```python
from build123d import *

# Parameters (mm, degrees)
SKETCH_1_W            = 100
SKETCH_1_H            = 50
EXTRUDE_1_DEPTH       = 15
HOLE_WIZARD_7_0_7_1_D = 7
CHAMFER_1_SIZE        = 3
SKETCH_6_W            = 2
SKETCH_6_H            = 30
CUT_EXTRUDE_1_DEPTH   = 113


with BuildPart() as part:
    # 草图1 → 凸台-拉伸1 (new body)
    with BuildSketch(Plane.XY):
        with Locations((50, 25)):
            Rectangle(SKETCH_1_W, SKETCH_1_H)
    extrude(amount=EXTRUDE_1_DEPTH)

    # Ø7.0 (7) 直径孔1 (through all)
    with Locations(Plane(origin=(0, 0, 0), x_dir=(-1, 0, 0), z_dir=(0, 0, -1))):
        with Locations((-10, 44), (-10, 6), (-90, 44), (-90, 6)):
            Hole(HOLE_WIZARD_7_0_7_1_D / 2)

    # 倒角1
    chamfer_1_edges = [part.edges().sort_by_distance(p)[0] for p in [
        (0, 50, 7.5),
        (100, 50, 7.5),
        (100, 0, 7.5),
        (0, 0, 7.5),
    ]]
    chamfer(chamfer_1_edges, length=CHAMFER_1_SIZE)

    # 草图6 → 切除-拉伸1 (cut)
    with BuildSketch(Plane.ZY):
        with Locations((1, 25)):
            Rectangle(SKETCH_6_W, SKETCH_6_H)
    extrude(amount=-CUT_EXTRUDE_1_DEPTH, mode=Mode.SUBTRACT)


solid = part.part
```
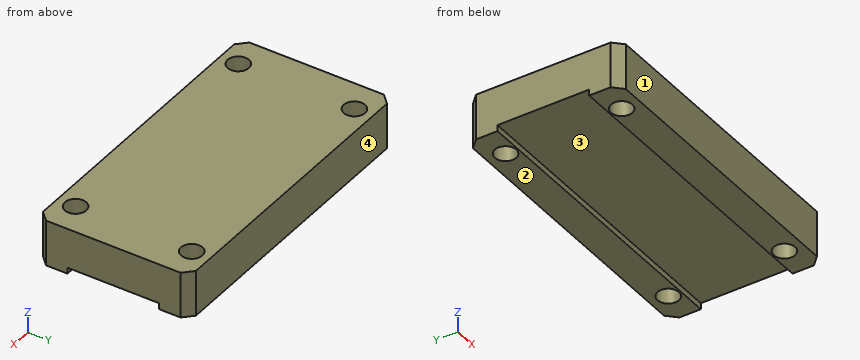
Model file for the job. Use its own axes, mm. Face numbers are marked on the shaded views. Coordinates: 2 decimals unless noted, no trailing zeros. Write each loop counter-clockwise with the first axis right and the second up, starting at its lowest first coordinate (ties: lowest second). Pieces come first, ordered by that corner, then holes. Notation, with made-up numbers: (-39.75, 17) - (-19.75, 17) arc R26 ccw to (-19.75, 38) - close; hole circle Ø6 at (24, 43). An arc over 180 degrees is marked (long way). One line per item, written item: value. Start each with the question number.
1. Slice it at D-D (x = 84). Write the cut outline in (y, z).
2. Mould opens along Y. For the marked faces 1, 2, 3 and 4 say: released by +Y, released by -Y, zero draft, split by the parting line, or undercut.
3. Slice it at B-B (y = 44). Write the cut outline in (x, z).
4. Slice it at C-C (z = 12.5). Write the cut outline in (x, y), plus the area to 3 significant figures.
5. Slice it at A-A (x = 10). Write the cut outline in (y, z), plus the area to 3 significant figures.
6. Probe line 1 (Y direction, x = 90, z = 11); line 2 (X direction, y = 7, z = 7.5); line 3 (X direction, y = 4.5, z = 2). List the from-to ranges inside material, lowest first. Write a range as from..to.
7. Flat gauge pin, fed straight in: pin 1 (9 mm diameter, centred on x = 63.5, y = 22, fed in from -Z). Where does the tip first touch, or does it go through?
Answers below:
1. outline: (0, 0) - (10, 0) - (10, 2) - (40, 2) - (40, 0) - (50, 0) - (50, 15) - (0, 15) - close
2. face 1: released by -Y
2. face 2: zero draft
2. face 3: undercut
2. face 4: released by +Y
3. outline: (0, 0) - (6.5, 0) - (6.5, 15) - (0, 15) - close; (13.5, 0) - (86.5, 0) - (86.5, 15) - (13.5, 15) - close; (93.5, 0) - (100, 0) - (100, 15) - (93.5, 15) - close
4. outline: (0, 3) - (3, 0) - (97, 0) - (100, 3) - (100, 47) - (97, 50) - (3, 50) - (0, 47) - close; hole circle Ø7 at (10, 6); hole circle Ø7 at (10, 44); hole circle Ø7 at (90, 6); hole circle Ø7 at (90, 44)
4. area: 4,830 mm^2
5. outline: (0, 0) - (2.5, 0) - (2.5, 15) - (0, 15) - close; (9.5, 0) - (10, 0) - (10, 2) - (40, 2) - (40, 0) - (40.5, 0) - (40.5, 15) - (9.5, 15) - close; (47.5, 0) - (50, 0) - (50, 15) - (47.5, 15) - close
5. area: 480 mm^2
6. line 1: y = 0..2.5, 9.5..40.5, 47.5..50
6. line 2: x = 0..6.65, 13.35..86.65, 93.35..100
6. line 3: x = 0..6.84, 13.16..86.84, 93.16..100
7. pin 1: stops at z = 2
